Build history of the part. All positions in model axes, mm. Face numbers are marked on the shaded views. A direction names the side the tool comes from. Round coordinates to 2 decimals unless told otherwise and drop trailing zeros. Write each loop counter-clockwise with the first axis right and the second up, starting at its lowest first coordinate (ties: lowest second). Pieces come first, ordered by that corner, then holes. Notation, with made-up numbers: (80, -7.5) -> (101, -7.5) arc R21 ccw to (101, 4.5) -> close; hole circle Ø7 at (26, -34.75). An arc over 180 degrees is marked (long way). Answer as CSV lines item,"result".
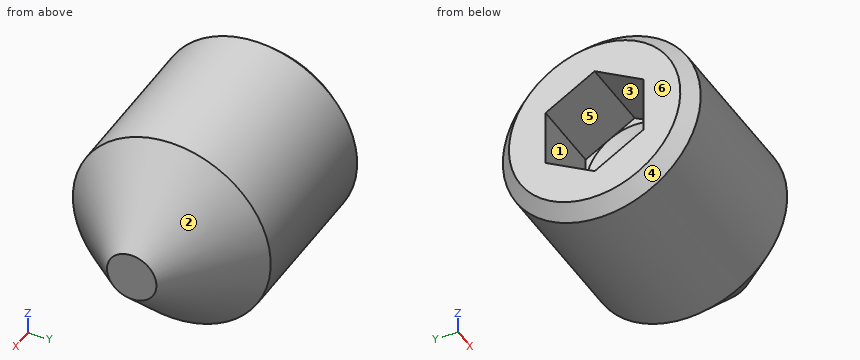
from build123d import *

# Parameters (mm, degrees)
CUT_EXTRUDE_1_DEPTH = 3


with BuildPart() as part:
    # 草图1 → Revolve 552 (revolve)
    with BuildSketch(Plane.XY, mode=Mode.PRIVATE) as revolve_552_sk:
        Polygon((0, 0), (10, 0), (10, 1), (7, 4), (0.536, 4), (0, 3.464), align=None)
    revolve(revolve_552_sk.sketch.rotate(Axis((-1.4104518, 0, 0), (1, 0, 0)), 90), axis=Axis((-1.4104518, 0, 0), (1, 0, 0)))

    # 草图2 → 切除-拉伸1 (cut)
    with BuildSketch(Plane.ZY):
        Polygon((2.29, 0), (1.145, 1.983198175), (-1.145, 1.983198175), (-2.29, 0), (-1.145, -1.983198175), (1.145, -1.983198175), align=None)
    extrude(amount=-CUT_EXTRUDE_1_DEPTH, mode=Mode.SUBTRACT)

    # 草图3 → 切除-旋转1 (revolve, cut)
    with BuildSketch(Plane.XY, mode=Mode.PRIVATE) as cut_revolve_1_sk:
        Polygon((3, 1.983198175), (4.145, 0), (3, 0), align=None)
    revolve(cut_revolve_1_sk.sketch.rotate(Axis((-0.121283255, 0, 0), (1, 0, 0)), 90), axis=Axis((-0.121283255, 0, 0), (1, 0, 0)), mode=Mode.SUBTRACT)


solid = part.part
1. Which spindle directions (+Z, -Z, +X, -X, +Y, -Y) get a long thin tool onto all of the face, cutting with end or side? Do the marked faces 1 and 2. Say none if no direction does.
Results found:
face 1,"-X"
face 2,"+X"
2. Probe line 1 along Z through (x, y) = (9, -0.25); line 2 along Z through (x, y) = (0.75, 0.5); line 3 along Y through (x, z) = (2, -0.25). List the from-to ranges inside material, lowest first.
Results found:
line 1,"z = -1.98 to 1.98"
line 2,"z = -3.97 to -2, 2 to 3.97"
line 3,"y = -3.99 to -1.98, 1.98 to 3.99"
3. Mould opens along Z. For the marked faces 3, 4, 5 and 6 say: +Z half, -Z half, draft (parallel to the pull), parting line (faces both ways), or undercut.
Results found:
face 3,"undercut"
face 4,"parting line"
face 5,"undercut"
face 6,"draft"
4. Drop flat-ended pins along their axis: pin 1 Ø2 at (x, z) = (7.5, 2) entering from +Y; pin 2 Ø2 at (y, z) = (2.5, 1.5) entering from +X; pin 3 Ø3 at (x, z) = (5.5, 2) entering from -Y. Give the stop position or say it passes through.
Results found:
pin 1,"stops at y = 3.84"
pin 2,"stops at x = 9.08"
pin 3,"stops at y = -3.97"
5. Cut at B-B, the plane x = 7.5. Write the cut outline in (y, z), then the cut area to 3 significant figures.
Results found:
outline,"circle Ø7 at (0, 0)"
area,"38.5 mm2"
6. Cut at A-A, the plane x = 5. Write the cut outline in (y, z).
Results found:
outline,"circle Ø8 at (0, 0)"
